Source: CAD feature listing. Evaluate the final solid. Frame: model axes, mm. Face numbers are marked on the shaded views. A direction names the side the tool comes from. Give positions to 0.01 mm unless a question says otherwise; leave off trailing zeros. Order: outer loops, then holes, each group sorted by start corner. A loop starts at its lowest first (then second) coordinate and runs counter-clockwise, first axis right, second up. Notation, with made-up numbers: (87.25, 45.25) - (107.25, 45.25) arc R14 cw to (107.25, 62.25) - close; hole circle Ø5 at (31.25, 62.5). An arc over 180 degrees is marked (long way). Answer as CSV lines item,"result".
```python
from build123d import *

# Parameters (mm, degrees)
SKETCH1_W                                            = 32
SKETCH1_H                                            = 15
BOSS_EXTRUDE1_DEPTH                                  = 10
CBORE_FOR_M5_HEXAGON_SOCKET_HEAD_CAP_SCR_D           = 5.5
CBORE_FOR_M5_HEXAGON_SOCKET_HEAD_CAP_SCR_DEPTH       = 12.4
CBORE_FOR_M5_HEXAGON_SOCKET_HEAD_CAP_SCR_CBORE_D     = 10
CBORE_FOR_M5_HEXAGON_SOCKET_HEAD_CAP_SCR_CBORE_DEPTH = 5.7
CBORE_FOR_M5_HEXAGON_SOCKET_HEAD_CAP_SCR_TIP         = 1.652366702
FILLET1_R                                            = 3


with BuildPart() as part:
    # Sketch1 → Boss-Extrude1 (new body)
    with BuildSketch(Plane.XY):
        Rectangle(SKETCH1_W, SKETCH1_H)
    extrude(amount=BOSS_EXTRUDE1_DEPTH)

    # CBORE for M5 Hexagon socket head cap screws1
    with Locations(Plane.XY.offset(10)):
        with Locations((7.5, 0), (-7.5, 0)):
            CounterBoreHole(CBORE_FOR_M5_HEXAGON_SOCKET_HEAD_CAP_SCR_D / 2, CBORE_FOR_M5_HEXAGON_SOCKET_HEAD_CAP_SCR_CBORE_D / 2, CBORE_FOR_M5_HEXAGON_SOCKET_HEAD_CAP_SCR_CBORE_DEPTH, depth=CBORE_FOR_M5_HEXAGON_SOCKET_HEAD_CAP_SCR_DEPTH)
            with Locations((0, 0, -(CBORE_FOR_M5_HEXAGON_SOCKET_HEAD_CAP_SCR_DEPTH + CBORE_FOR_M5_HEXAGON_SOCKET_HEAD_CAP_SCR_TIP / 2))):  # 118° drill point
                Cone(0, CBORE_FOR_M5_HEXAGON_SOCKET_HEAD_CAP_SCR_D / 2, CBORE_FOR_M5_HEXAGON_SOCKET_HEAD_CAP_SCR_TIP, mode=Mode.SUBTRACT)

    # Fillet1
    fillet1_edges = [part.edges().sort_by_distance(p)[0] for p in [
        (16, -7.5, 5),
        (-16, -7.5, 5),
        (-16, 7.5, 5),
        (16, 7.5, 5),
    ]]
    fillet(fillet1_edges, radius=FILLET1_R)


solid = part.part
```
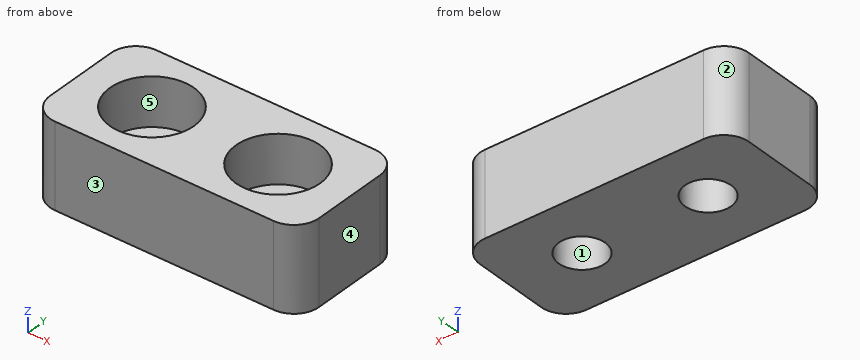
(1) Contact query for flat-ended pins moving along their axis: pin 1 (4.5 mm diameter, centred on x = 7.5, y = 0, fed in from -Z); pin 2 (6 mm diameter, centred on x = 7.5, y = 0, fed in from +Z). Output: stop coordinate, or through.
Completed:
pin 1,"through"
pin 2,"z = 4.3"
(2) Access query for the marked faces 4 and 5. Directions: +Z, -Z, +X, -X, +Y, -Y. A direction counts if a zero-diameter tool reaches every point of the face in a straight line with its end or side. Return the directions, or none.
Completed:
face 4,"+Z, -Z, +X, +Y, -Y"
face 5,"+Z"
(3) Cut plane A-A (y = 0). Return loops of the section in (x, z).
Completed:
outline,"(-16, 0) - (-10.25, 0) - (-10.25, 4.3) - (-12.5, 4.3) - (-12.5, 10) - (-16, 10) - close; (-4.75, 0) - (4.75, 0) - (4.75, 4.3) - (2.5, 4.3) - (2.5, 10) - (-2.5, 10) - (-2.5, 4.3) - (-4.75, 4.3) - close; (10.25, 0) - (16, 0) - (16, 10) - (12.5, 10) - (12.5, 4.3) - (10.25, 4.3) - close"
(4) Cut plane D-D (z = 2.75). Return loops of the section in (x, y).
Completed:
outline,"(-16, -4.5) arc R3 ccw to (-13, -7.5) - (13, -7.5) arc R3 ccw to (16, -4.5) - (16, 4.5) arc R3 ccw to (13, 7.5) - (-13, 7.5) arc R3 ccw to (-16, 4.5) - close; hole circle Ø5.5 at (-7.5, 0); hole circle Ø5.5 at (7.5, 0)"
(5) Ray query, line 1 (Y direction, x = 7.5, z = 8.5); line 2 (Y direction, x = -7.5, z = 2.25); line 3 (X direction, y = 3.25, z = 6). Return the intervals inside material, ascending. Write a range as from..to.
Completed:
line 1,"-7.5..-5, 5..7.5"
line 2,"-7.5..-2.75, 2.75..7.5"
line 3,"-16..-11.3, -3.7..3.7, 11.3..16"
(6) Mould query, pull axis X, two halves, no side actions, for the marked faces 1, 2 and 3. Classes: released by +X, released by -X, zero draft, split by the parting line, or undercut.
Completed:
face 1,"undercut"
face 2,"released by -X"
face 3,"zero draft"
(7) Cut plane B-B (z = 8.5). Return loops of the section in (x, y).
Completed:
outline,"(-16, -4.5) arc R3 ccw to (-13, -7.5) - (13, -7.5) arc R3 ccw to (16, -4.5) - (16, 4.5) arc R3 ccw to (13, 7.5) - (-13, 7.5) arc R3 ccw to (-16, 4.5) - close; hole circle Ø10 at (-7.5, 0); hole circle Ø10 at (7.5, 0)"
(8) Cut plane C-C (x = 7). Return loops of the section in (y, z), then the cut area to 3 significant figures.
Completed:
outline,"(-7.5, 0) - (-2.7, 0) - (-2.7, 4.3) - (-4.97, 4.3) - (-4.97, 10) - (-7.5, 10) - close; (2.7, 0) - (7.5, 0) - (7.5, 10) - (4.97, 10) - (4.97, 4.3) - (2.7, 4.3) - close"
area,"70.0 mm²"
